Could you check a few things on this model? Use its own coordinates, in mm. Coordinates: 2 decimals unless noted, no trailing zeros. Write each loop counter-clockwise with the first axis right and the second up, starting at its lowest first coordinate (ties: lowest second). Pieces come first, ordered by that corner, then holes.
Item 1: I want a section at B-B on x = -56. Please give me the cut outline in (y, z), then the cut area to 3 significant figures.
Item 2: If I drill on probe 1 along X at (y, z) = (28.5, 0.9); probe 2 along Y at (x, z) = (43.15, -0.4); probe 3 along Y at (x, z) = (-56, -0.75), over which ranges is the centre line in solid material (lowest first)?
Item 3: I want a section at A-A on y = -23.85. Please give me the cut outline in (x, z), then the cut area to 3 significant figures.
Item 4: For P1, Ø3, axis at x = -56, y = 28.75, coming from the +Z side, with a flat end and sliding along its axis, tell me the tip position at first contact or that it passes through.
Item 5: Thinking about a two-plate mould opening in X: for faces 1 (the flat face through (-61, 0, 0)), 2 (the flat face through (-1, -32.75, 0)), 3 (the cylindrical face through (45.296, -23.174, -0.028)), which applies, +X half, -X half, draft (parallel to the pull), parting line (faces both ways), or undercut?
Item 6: I want a section at C-C on y = 28.75. Please give me the cut outline in (x, z).
from build123d import *

# Parameters (mm, degrees)
SKETCH_1_W      = 122
SKETCH_1_H      = 65.5
SKETCH_1_R      = 1.75
SKETCH_1_R_2    = 2.25
EXTRUDE_1_DEPTH = 2
FILLET_1_R      = 2


with BuildPart() as part:
    # 草图1 → 凸台-拉伸1 (new, symmetric)
    with BuildSketch(Plane.XY):
        Rectangle(SKETCH_1_W, SKETCH_1_H)
        with Locations((-56, 28.75)):
            Circle(SKETCH_1_R, mode=Mode.SUBTRACT)
        with Locations((-45, 8.15)):
            Circle(SKETCH_1_R_2, mode=Mode.SUBTRACT)
        with Locations((45, 8.15)):
            Circle(SKETCH_1_R_2, mode=Mode.SUBTRACT)
        with Locations(Location((56, 28.75, 0), (0, 0, 180))):
            Circle(SKETCH_1_R, mode=Mode.SUBTRACT)
        with Locations((-43.15, -23.85)):
            Circle(SKETCH_1_R_2, mode=Mode.SUBTRACT)
        with Locations((43.15, -23.85)):
            Circle(SKETCH_1_R_2, mode=Mode.SUBTRACT)
    extrude(amount=EXTRUDE_1_DEPTH, both=True)

    # 圆角1
    fillet_1_edges = [part.edges().sort_by_distance(p)[0] for p in [
        (61, -32.75, 0),
        (-61, -32.75, 0),
        (-61, 32.75, 0),
        (61, 32.75, 0),
    ]]
    fillet(fillet_1_edges, radius=FILLET_1_R)


solid = part.part
Response values:
1. outline: (-32.75, -2) - (27, -2) - (27, 2) - (-32.75, 2) - close; (30.5, -2) - (32.75, -2) - (32.75, 2) - (30.5, 2) - close
1. area: 248 mm2
2. probe 1: x = -61 to -57.73, -54.27 to 54.27, 57.73 to 61
2. probe 2: y = -32.75 to -26.1, -21.6 to 6.87, 9.43 to 32.75
2. probe 3: y = -32.75 to 27, 30.5 to 32.75
3. outline: (-61, -2) - (-45.4, -2) - (-45.4, 2) - (-61, 2) - close; (-40.9, -2) - (40.9, -2) - (40.9, 2) - (-40.9, 2) - close; (45.4, -2) - (61, -2) - (61, 2) - (45.4, 2) - close
3. area: 452 mm2
4. P1: passes through
5. face 1: -X half
5. face 2: draft
5. face 3: undercut
6. outline: (-61, -2) - (-57.75, -2) - (-57.75, 2) - (-61, 2) - close; (-54.25, -2) - (54.25, -2) - (54.25, 2) - (-54.25, 2) - close; (57.75, -2) - (61, -2) - (61, 2) - (57.75, 2) - close
